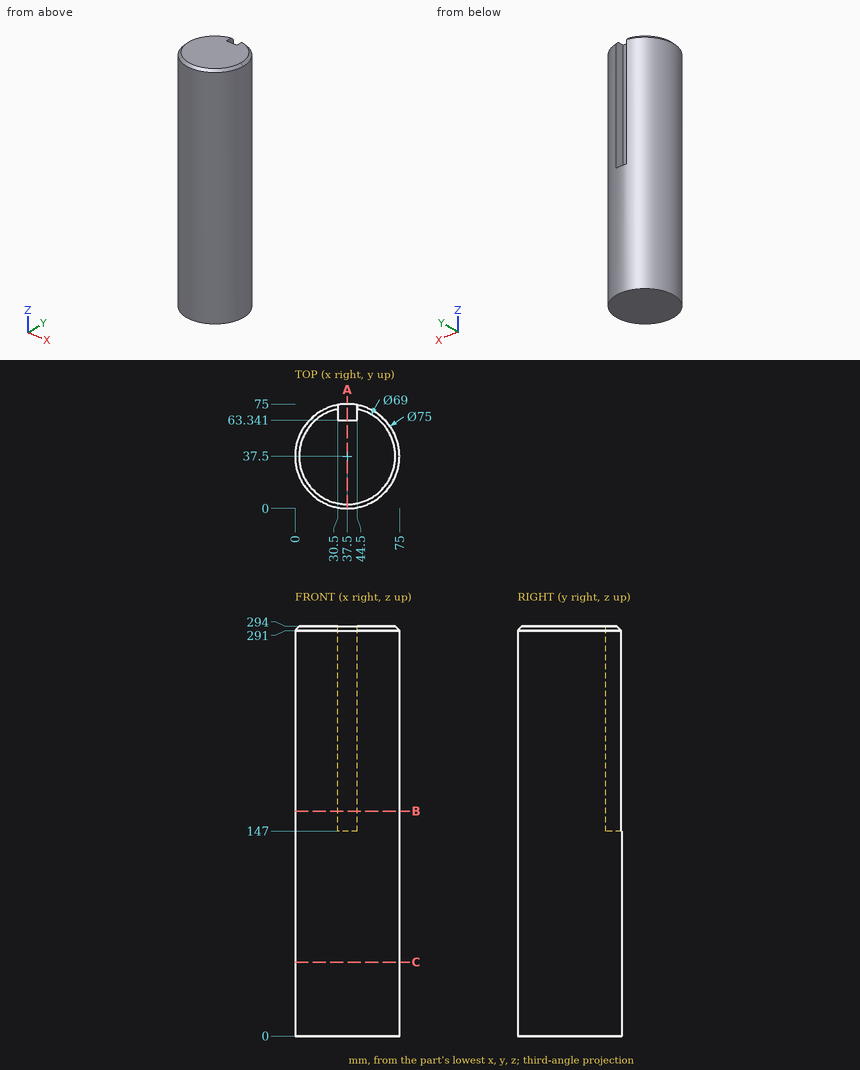
Part print with two shaded views. Sizes in mm from the minimum x, y, z corner. Coordinates: 2 decimals unless noted, no trailing zeros. Write each loop counter-clockwise with the first axis right and the second up, starting at its lowest first coordinate (ties: lowest second). Pieces come first, ordered by that corner, then holes. Notation, with made-up numbers: (-6.75, 55.25) - (5.25, 55.25) arc R18 cw to (5.25, 77.25) - close; hole circle Ø3 at (-14, -28.75). An arc over 180 degrees is marked (long way). Use a Markdown table: item, result. Add a question column.
Item 1: Drill centre lines: line 1 along Z through (x, y) = (43, 68.5); line 2 along X through (y, z) = (69.5, 179.5); line 3 along X through (y, z) = (16, 184.5) (1 decimal). Where is each one in solid material? Low to high.
Item 2: Band-saw the part on B-B, the plane z = 161.5. Write the cut outline in (x, y).
Item 3: Drop flat-ended pins along their axis: pin 1 (2 mm diameter, centred on y = 57, z = 123.5, fed in from -X); pin 2 (12 mm diameter, centred on x = 59, z = 229.5, fed in from -Y); pin 3 (2 mm diameter, centred on x = 33.5, z = 253.5, fed in from +Y). Give the stop position or say it passes through.
Item 4: Band-saw the part on C-C, the plane z = 53. Write the cut outline in (x, y).
Item 5: Band-saw the part on A-A, the plane x = 37.5. Write the cut outline in (y, z), and give its area (3 significant figures).
A:
| question | item | result |
|---|---|---|
| 1 | line 1 | z = 0 to 147 |
| 1 | line 2 | x = 17.95 to 30.5, 44.5 to 57.05 |
| 1 | line 3 | x = 6.8 to 68.2 |
| 2 | outline | (30.5, 63.34) - (30.5, 74.34) arc R37.5 ccw (long way) to (44.5, 74.34) - (44.5, 63.34) - close |
| 3 | pin 1 | stops at x = 4.88 |
| 3 | pin 2 | stops at y = 3.35 |
| 3 | pin 3 | stops at y = 63.34 |
| 4 | outline | circle Ø75 at (37.5, 37.5) |
| 5 | outline | (0, 0) - (75, 0) - (75, 147) - (63.34, 147) - (63.34, 294) - (3, 294) - (0, 291) - close |
| 5 | area | 20,300 mm² |
